from build123d import *

# Parameters (mm, degrees)
SKETCH1_R           = 7
BOSS_EXTRUDE1_DEPTH = 3


with BuildPart() as part:
    # Sketch1 → Boss-Extrude1 (new body)
    with BuildSketch(Plane(origin=(0, 0, 0), x_dir=(1, 0, 0), z_dir=(0, 1, 0))):
        with BuildLine():
            Line((-22.5, 100), (22.5, 100))
            Line((22.5, 100), (22.5, 20))
            Line((22.5, 20), (8.749140244, -4.842782774))
            ThreePointArc((8.749140244, -4.842782774), (0, -10), (-8.749140244, -4.842782774))
            Line((-8.749140244, -4.842782774), (-22.5, 20))
            Line((-22.5, 20), (-22.5, 100))
        make_face()
        with Locations(Location((0, 0, 0), (0, 0, 270))):
            Circle(SKETCH1_R, mode=Mode.SUBTRACT)
        with BuildLine():
            Line((-15.5, 27.5), (-15.5, 92.5))
            ThreePointArc((-15.5, 92.5), (-12.5, 95.5), (-9.5, 92.5))
            Line((-9.5, 92.5), (-9.5, 27.5))
            ThreePointArc((-9.5, 27.5), (-12.5, 24.5), (-15.5, 27.5))
        make_face(mode=Mode.SUBTRACT)
        with BuildLine():
            Line((15.5, 27.5), (15.5, 92.5))
            ThreePointArc((15.5, 92.5), (12.5, 95.5), (9.5, 92.5))
            Line((9.5, 92.5), (9.5, 27.5))
            ThreePointArc((9.5, 27.5), (12.5, 24.5), (15.5, 27.5))
        make_face(mode=Mode.SUBTRACT)
    extrude(amount=BOSS_EXTRUDE1_DEPTH)


solid = part.part
Read the model definition and answer for the solid it produces. Units are mm, in the model's axes. A direction names the side the tool comes from. Give positions to 0.01 mm unless a question says otherwise; leave off trailing zeros. Write each loop counter-clockwise with the first axis right and the second up, starting at its lowest first coordinate (ties: lowest second). Pieces come first, ordered by that corner, then holes. Notation, with made-up numbers: M 89,2 L 120,2 A22 cw 120,19 Z; hole C 47,37 d2. An arc over 180 degrees is marked long. One line per item, written item: value. Start each with the question number.
(1) A flat-ended cylindrical pin translates along its axis: pin 1 Ø3 at (x, z) = (-10.5, -39) entering from -Y. Find the tip coordinate at first contact, or state that the pin passes through.
(2) A tool of negligible diameter and unlimited length cuts with its end or side. For faces 1 (the cylindrical face through (12.6, 1.5, -95.5)), 2 (the flat face through (0, 3, -46)), from which of +Z, -Z, +X, -X, +Y, -Y can it reach the whole face along a straight path? Write none if from no direction.
(3) Find section B-B (x = 0). Determine the outline of the cut face in (y, z), plus the area to 3 significant figures.
(4) Find section A-A (y = 2.3). Determine the outline of the cut face in (x, z), plus the area to 3 significant figures.
(5) Determine the mould class of faces 3 (the flat face through (-15.528, 1.479, -7.405)), 4 (the cylindrical face through (-12.6, 1.5, -95.5)), 5 (the cylindrical face through (0, 1, 10)) for opening direction X: pulls with the +X half, pulls with the -X half, needs draft (parallel to the pull), parting line crosses it, or undercut.
(6) Find the intervals of material crossed by line 1 (X direction, y = 1.1, z = -40.5); line 2 (Z direction, x = 12, y = 0.3); line 3 (X direction, y = 1.4, z = 0), in increasing order.
(7) Find section C-C (z = -31). Determine the outline of the cut face in (x, y).
(8) Find section D-D (z = 0). Determine the outline of the cut face in (x, y).
Results below:
1. pin 1: stops at y = 0
2. face 1: +Y, -Y
2. face 2: +Z, -Z, +X, -X, +Y
3. outline: M 0,-100 L 3,-100 L 3,-7 L 0,-7 Z; M 0,7 L 3,7 L 3,10 L 0,10 Z
3. area: 288 mm^2
4. outline: M -22.5,-100 L 22.5,-100 L 22.5,-20 L 8.75,4.84 A10 ccw -8.75,4.84 L -22.5,-20 Z; hole M -15.5,-92.5 A3 ccw -9.5,-92.5 L -9.5,-27.5 A3 ccw -15.5,-27.5 Z; hole C 0,0 d14; hole M 9.5,-92.5 A3 ccw 15.5,-92.5 L 15.5,-27.5 A3 ccw 9.5,-27.5 Z
4. area: 3,450 mm^2
5. face 3: pulls with the -X half
5. face 4: undercut
5. face 5: parting line crosses it
6. line 1: x = -22.5 to -15.5, -9.5 to 9.5, 15.5 to 22.5
6. line 2: z = -100 to -95.46, -24.54 to -1.03
6. line 3: x = -11.43 to -7, 7 to 11.43
7. outline: M -22.5,0 L -15.5,0 L -15.5,3 L -22.5,3 Z; M -9.5,0 L 9.5,0 L 9.5,3 L -9.5,3 Z; M 15.5,0 L 22.5,0 L 22.5,3 L 15.5,3 Z
8. outline: M -11.43,0 L -7,0 L -7,3 L -11.43,3 Z; M 7,0 L 11.43,0 L 11.43,3 L 7,3 Z
